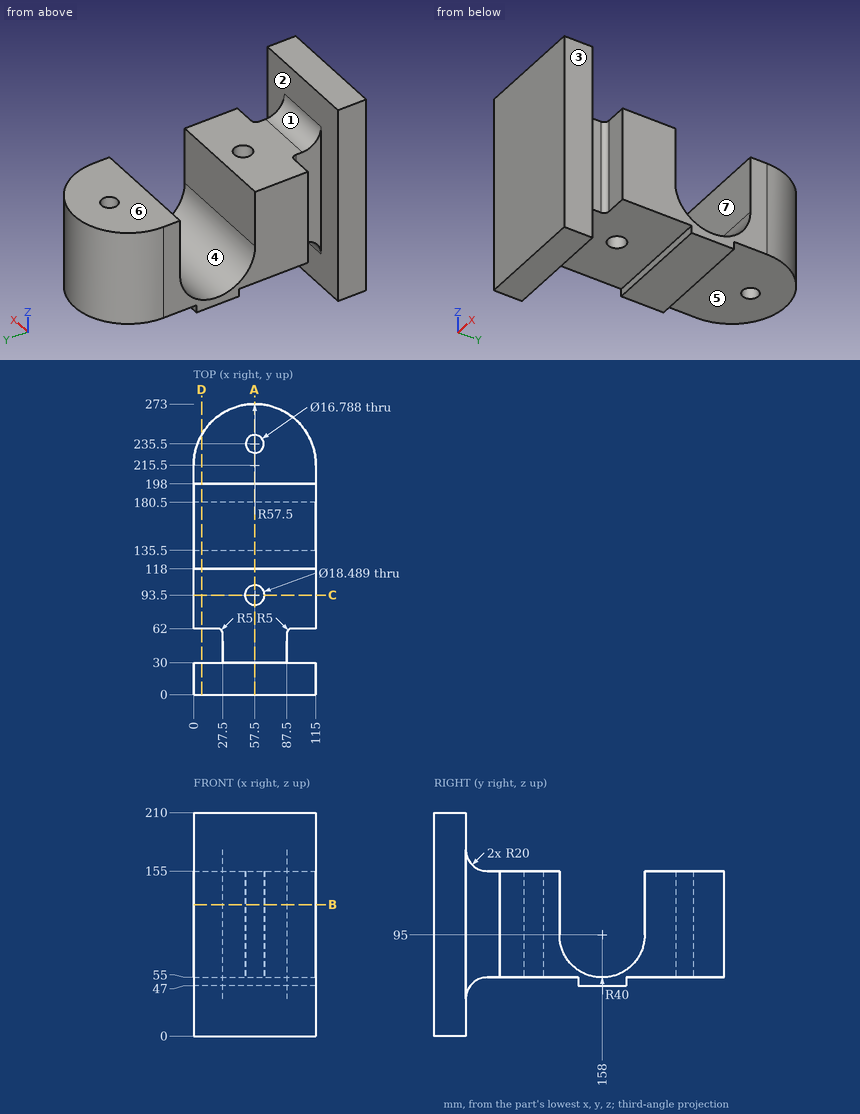
Check sheet for the drawn part. Datum: minimum x, y, z corner. Units: mm. A direction names the side the tool comes from. Round coordinates to 2 decimals unless told otherwise and drop trailing zeros. Loops run counter-clockwise (first coordinate to the right, second up) from the corner with the lowest first, then second, coordinate; pieces in that order, holes last.
Item 1: Gauge pin test, flat ends, axial feed: pin 1 (10 mm diameter, centred on x = 35.5, z = 63, fed in from +Y); pin 2 (1 mm diameter, centred on y = 56.5, z = 128, fed in from -X); pin 3 (15 mm diameter, centred on x = 57.5, y = 93.5, fed in from -Z); pin 4 (4 mm diameter, centred on x = 50.5, y = 55, fed in from +Z). Record the tip position at first contact, or that the pin passes through.
Item 2: Access from +Z, -Z, +X, -X, +Y, -Y to the whole of each face (thin tool, end or side, straight path). Record for the marked faces 5, 6 and 7.
Item 3: Cross-section at B-B on z = 123.5. Record the boundary of the cut face in (x, y), then the cut area to 3 significant figures.
Item 4: Thickness scan on line 1 (Y direction, x = 57.5, z = 131.5); line 2 (Y direction, x = 103, z = 109); line 3 (Y direction, x = 57, z = 71). Record the ranges inside material, lowest first.
Item 5: Cross-section at D-D on x = 7.5. Record the boundary of the cut face in (y, z).
Item 6: Mould release check, pull along Y, two halves, no side actions. Record for the marked faces 1, 2, 3 and 4: pulls with the +Y half, pulls with the -Y half, needs draft (parallel to the pull), parting line crosses it, or undercut.
Item 7: Cross-section at C-C on y = 93.5. Record the boundary of the cut face in (x, z), then the cut area to 3 significant figures.
Item 8: Cross-section at A-A on x = 57.5. Record the boundary of the cut face in (y, z).
Answer sheet:
1. pin 1: stops at y = 270.43
1. pin 2: stops at x = 27.5
1. pin 3: passes through
1. pin 4: stops at z = 155
2. face 5: -Z, +X, -X, +Y
2. face 6: +Z, +X, -X, +Y
2. face 7: +Z, +X, -X
3. outline: (0, 0) - (115, 0) - (115, 30) - (87.5, 30) - (87.5, 57) arc R5 cw to (92.5, 62) - (115, 62) - (115, 118) - (0, 118) - (0, 62) - (22.5, 62) arc R5 cw to (27.5, 57) - (27.5, 30) - (0, 30) - close; (0, 198) - (115, 198) - (115, 215.5) arc R57.5 ccw to (0, 215.5) - close; hole circle Ø18.49 at (57.5, 93.5); hole circle Ø16.79 at (57.5, 235.5)
3. area: 18,500 mm2
4. line 1: y = 0 to 84.26, 102.74 to 118, 198 to 227.11, 243.89 to 273
4. line 2: y = 0 to 30, 62 to 118, 198 to 250.66
4. line 3: y = 0 to 84.27, 102.73 to 126, 190 to 227.12, 243.88 to 273
5. outline: (0, 0) - (30, 0) - (30, 210) - (0, 210) - close; (62, 55) - (135.5, 55) - (135.5, 47) - (180.5, 47) - (180.5, 55) - (243.89, 55) - (243.89, 155) - (198, 155) - (198, 95) arc R40 cw to (118, 95) - (118, 155) - (62, 155) - close
6. face 1: pulls with the +Y half
6. face 2: undercut
6. face 3: needs draft
6. face 4: undercut
7. outline: (0, 55) - (48.26, 55) - (48.26, 155) - (0, 155) - close; (66.74, 55) - (115, 55) - (115, 155) - (66.74, 155) - close
7. area: 9,650 mm2
8. outline: (0, 0) - (30, 0) - (30, 35) arc R20 cw to (50, 55) - (84.26, 55) - (84.26, 155) - (50, 155) arc R20 cw to (30, 175) - (30, 210) - (0, 210) - close; (102.74, 55) - (135.5, 55) - (135.5, 47) - (180.5, 47) - (180.5, 55) - (227.11, 55) - (227.11, 155) - (198, 155) - (198, 95) arc R40 cw to (118, 95) - (118, 155) - (102.74, 155) - close; (243.89, 55) - (273, 55) - (273, 155) - (243.89, 155) - close
